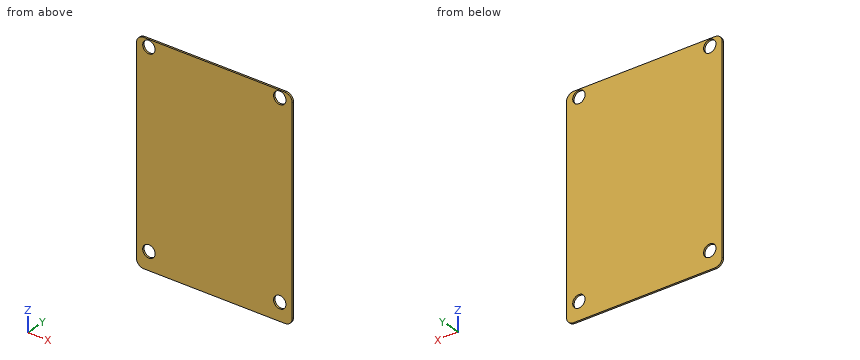
from build123d import *

# Parameters (mm, degrees)
SKETCH1_W                      = 139.7
SKETCH1_H                      = 190.5
BOSS_EXTRUDE1_DEPTH            = 1.5748
FILLET1_R                      = 6.35
F_7_16_0_4375_DIAMETER_HOLE1_D = 11.1125
LPATTERN1_COUNT                = 2
LPATTERN1_PITCH                = 168.275
LPATTERN1_COUNT_DIR2           = 2
LPATTERN1_PITCH_DIR2           = 117.475


with BuildPart() as part:
    # Sketch1 → Boss-Extrude1 (new body)
    with BuildSketch(Plane(origin=(0, 0, 0), x_dir=(1, 0, 0), z_dir=(0, 1, 0))):
        with Locations((0, 4.7625)):
            Rectangle(SKETCH1_W, SKETCH1_H)
    extrude(amount=BOSS_EXTRUDE1_DEPTH)

    # Fillet1
    fillet1_edges = [part.edges().sort_by_distance(p)[0] for p in [
        (-69.85, 0.7874, -100.0125),
        (69.85, 0.7874, -100.0125),
        (69.85, 0.7874, 90.4875),
        (-69.85, 0.7874, 90.4875),
    ]]
    fillet(fillet1_edges, radius=FILLET1_R)

    # 7/16 (0.4375) Diameter Hole1 (through all)
    with Locations(Plane(origin=(0, 1.5748, 0), x_dir=(1, 0, 0), z_dir=(0, 1, 0))):
        with Locations((-58.738, 84.1375)):
            f_7_16_0_4375_diameter_hole1 = Hole(F_7_16_0_4375_DIAMETER_HOLE1_D / 2)

    # LPattern1: 7_16 _0.4375_ Diameter Hole1 2 × 2
    with Locations(*[(j * LPATTERN1_PITCH_DIR2, 0, i * LPATTERN1_PITCH) for i in range(LPATTERN1_COUNT) for j in range(LPATTERN1_COUNT_DIR2) if (i, j) != (0, 0)]):
        add(f_7_16_0_4375_diameter_hole1, mode=Mode.SUBTRACT)


solid = part.part
Geometry: final body of the model. Coordinates: model frame, mm. Give positions to 0.01 mm unless a question says otherwise; leave off trailing zeros. Write each loop counter-clockwise with the first axis right and the second up, starting at its lowest first coordinate (ties: lowest second). Pieces come first, ordered by that corner, then holes.
(1) Ray query, line 1 (X direction, y = 0.4, z = -84.5); line 2 (Z direction, x = 54, y = 0.7). Return the intervals inside material, ascending.
(2) First-contact query: P1, Ø13, axis at x = -58.74, z = -84.14, coming from the -Y side. Flat tip, straight axial feed; report the tip coordinate or a pass-through.
(3) Cut plane A-A, the plane y = 0.55. Return loops of the section in (x, z), then the cut area to 3 significant figures.
Values follow:
1. line 1: x = -69.85 to -64.28, -53.19 to 53.19, 64.28 to 69.85
1. line 2: z = -100.01 to -87.04, -81.23 to 81.23, 87.04 to 90.49
2. P1: stops at y = 0
3. outline: (-69.85, -93.66) arc R6.35 ccw to (-63.5, -100.01) - (63.5, -100.01) arc R6.35 ccw to (69.85, -93.66) - (69.85, 84.14) arc R6.35 ccw to (63.5, 90.49) - (-63.5, 90.49) arc R6.35 ccw to (-69.85, 84.14) - close; hole circle Ø11.11 at (-58.74, -84.14); hole circle Ø11.11 at (-58.74, 84.14); hole circle Ø11.11 at (58.74, -84.14); hole circle Ø11.11 at (58.74, 84.14)
3. area: 26,200 mm2
